Build history of the part. All positions in model axes, mm. Face numbers are marked on the shaded views. A direction names the side the tool comes from. Round coordinates to 2 decimals unless told otherwise and drop trailing zeros. Write each loop counter-clockwise with the first axis right and the second up, starting at its lowest first coordinate (ties: lowest second). Pieces come first, ordered by that corner, then holes. Notation, with made-up numbers: M 54.25,19 L 102.25,19 A23 ccw 102.25,49 Z; hole C -20,-27.75 d4. An arc over 180 degrees is marked long. Write item = value, one per line.
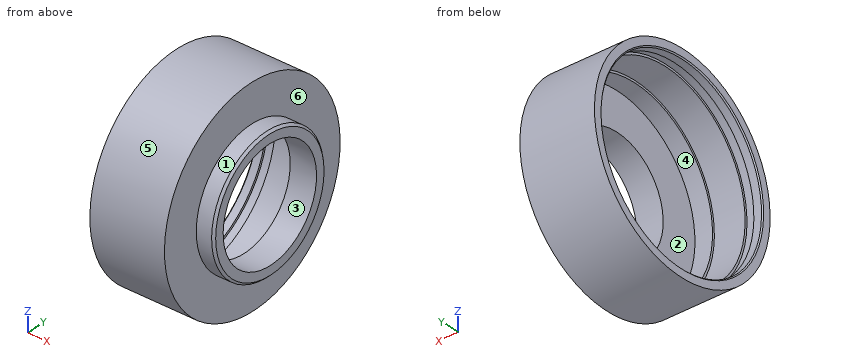
from build123d import *

# Parameters (mm, degrees)
CHAMFER_1_SIZE = 0.25
CHAMFER_2_SIZE = 0.5


with BuildPart() as part:
    # 草图1 → 旋转1 (revolve)
    with BuildSketch(Plane.XY, mode=Mode.PRIVATE) as revolve_1_sk:
        Polygon((2.179589421, 21.5), (4.179589421, 21.5), (4.179589421, 22), (6.179589421, 22), (6.179589421, 21.5), (13.179589421, 21.5), (13.179589421, 21), (17.179589421, 21), (17.179589421, 12.5), (23.179589421, 12.5), (23.179589421, 15), (19.179589421, 15), (19.179589421, 23.5), (2.179589421, 23.5), align=None)
    revolve(revolve_1_sk.sketch.rotate(Axis((0, 0, 0), (1, 0, 0)), 90), axis=Axis((0, 0, 0), (1, 0, 0)))

    # 倒角1
    chamfer_1_edges = [part.edges().sort_by_distance(p)[0] for p in [
        (2.179589421, 0, -21.5),
    ]]
    chamfer(chamfer_1_edges, length=CHAMFER_1_SIZE)

    # 倒角2
    chamfer_2_edges = [part.edges().sort_by_distance(p)[0] for p in [
        (23.179589421, 0, -15),
    ]]
    chamfer(chamfer_2_edges, length=CHAMFER_2_SIZE)


solid = part.part
1. Flat gauge pins, fed straight in: pin 1 (4 mm diameter, centred on x = 17, y = -13, fed in from -Z); pin 2 (13 mm diameter, centred on y = -5.5, z = -2.5, fed in from -X); pin 3 (8 mm diameter, centred on y = 14, z = 14.5, fed in from +X); pin 4 (22.5 mm diameter, centred on y = 0, z = 0, fed in from +X). Where does each tip first touch, or does it go through?
Responses:
pin_1 = -20.77
pin_2 = 17.18
pin_3 = 19.18
pin_4 = through
2. Band-saw the part on C-C (x = 11). List the corners of the cut face in (y, z), plus the area to 3 significant figures.
Responses:
outline = C 0,0 d47; hole C 0,0 d43
area = 283 mm²
3. Tool access for the marked faces 1, 2 and 3: list every direction of +Z, -Z, +X, -X, +Y, -Y with a clear straight run to the whole face (end or side of a thin tool).
Responses:
face_1 = +X
face_2 = -X
face_3 = +X, -X
4. Probe probe 1 along Y at (x, z) = (13, -0.5); probe 2 along Y at (x, z) = (14.7, 0); probe 3 along X at (y, z) = (-19.5, 11.5). List the from-to ranges inside material, lowest first.
Responses:
probe_1 = -23.49 to -21.49, 21.49 to 23.49
probe_2 = -23.5 to -21, 21 to 23.5
probe_3 = 2.18 to 19.18
5. Band-saw the part on D-D (x = 14). List the corners of the cut face in (y, z).
Responses:
outline = C 0,0 d47; hole C 0,0 d42
6. Mould opens along Y. For the marked faces 4, 5 and 6 say: pulls with the +Y half, pulls with the -Y half, needs draft (parallel to the pull), parting line crosses it, or undercut.
Responses:
face_4 = undercut
face_5 = parting line crosses it
face_6 = needs draft
